Here's the drawing with two shaded views (mm, measured from the low corner). I have some questions. Coordinates: 2 decimals unless noted, no trailing zeros. Write each loop counter-clockwise with the first axis right and the second up, starting at its lowest first coordinate (ties: lowest second). Pieces come first, ordered by that corner, then holes. Notation, with made-up numbers: (48.5, 81.5) -> (90.5, 81.5) arc R26 ccw to (90.5, 118.5) -> close; hole circle Ø1 at (-15, -6.5). An arc over 180 degrees is marked (long way). Put each result on its own line as item: value. Start each with the question number.
Item 1: I want a section at A-A, the plane z = 220. List the corners of the cut face in (x, y) for me.
Item 2: I want a section at B-B, the plane y = 322. List the corners of the cut face in (x, z) for me.
Item 3: For pin 1 (9 mm diameter, centred on x = 185, z = 370, fed in from +Y); pin 2 (1.5 mm diameter, centred on y = 151, z = 108.5, fed in from +X); pin 3 (2 mm diameter, centred on x = 331, z = 160, fed in from +Y), each with a flat end and sliding along its axis, tell me the tip position at first contact or that it passes through.
Item 4: I need wall thicknesses on line 1 (X direction, y = 3, z = 70); line 2 (X direction, y = 3.5, z = 220); line 3 (X direction, y = 219, z = 263.5). Which ranges of each line are inside material? Lowest first, please. Write a range as [from, to].
Item 5: If we mould it in two halves opening along Y, with no side actions, what happens to the marked faces 1, 2 and 3? For each: released by +Y, released by -Y, zero draft, split by the parting line, or undercut.
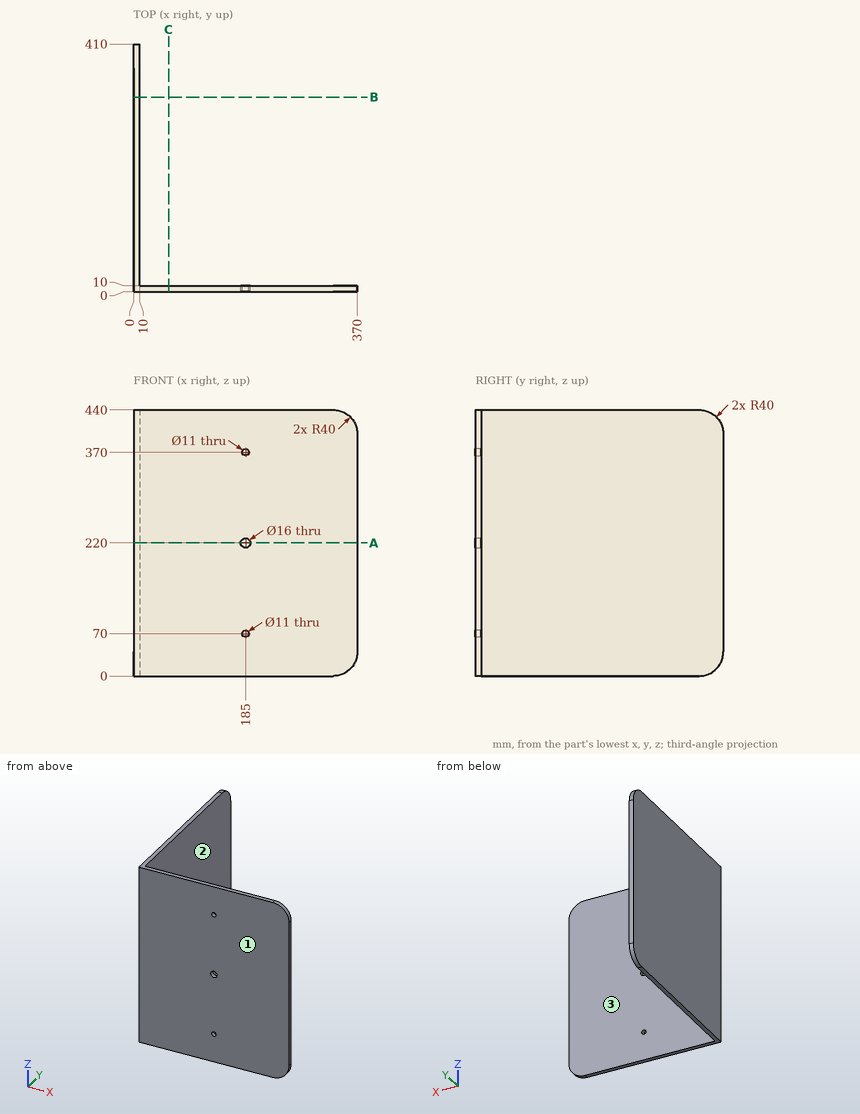
Calculated:
1. outline: (0, 0) -> (177, 0) -> (177, 10) -> (10, 10) -> (10, 410) -> (0, 410) -> close; (193, 0) -> (370, 0) -> (370, 10) -> (193, 10) -> close
2. outline: (0, 0) -> (10, 0) -> (10, 440) -> (0, 440) -> close
3. pin 1: passes through
3. pin 2: stops at x = 10
3. pin 3: stops at y = 10
4. line 1: x = [0, 179.5], [190.5, 370]
4. line 2: x = [0, 177], [193, 370]
4. line 3: x = [0, 10]
5. face 1: released by -Y
5. face 2: zero draft
5. face 3: released by +Y
